The listing builds one solid part. Answer for the finished solid, in the listing's coordinates (mm). Face numbers are marked on the shaded views. Give positions to 0.01 mm unless a question says otherwise; leave off trailing zeros. Loops run counter-clockwise (first coordinate to the right, second up) from the corner with the lowest first, then second, coordinate; pieces in that order, holes last. Notation, with made-up numbers: M 69,17 L 76,17 A24 cw 76,56 Z; hole C 87,39.25 d2. An arc over 180 degrees is marked long. One line per item, written item: value. Start each with the question number.
Q1. A flat-ended cylindrical pin translates along its axis: pin 1 (4 mm diameter, centred on x = -9, y = 6.5, fed in from +Z). Find the tip coordinate at first contact, or state that the pin passes through.
Q2. A cutting plane is placed at D-D, the plane z = 3.15. Determine the outline of the cut face in (x, y) (3 decimals), and give its area (3 significant figures).
Q3. A cutting plane is placed at C-C, the plane y = 14. Determine the outline of the cut face in (x, z).
Q4. A cutting plane is placed at A-A, the plane y = 0. Determine the outline of the cut face in (x, z) (3 decimals).
Q5. Consider L1, parallel to Y at x = 0, z = 1.1 (3 decimals); L2, parallel to Y at x = 0, z = 3.2 (3 decimals); L3, parallel to X at y = 6, z = 1.55. Determine where each line is inside the solid, lowest interval first.
Q6. The mould has two halves that part along X. Classify the marked faces 1, 2 and 3: +X half, -X half, draft (parallel to the pull), parting line (faces both ways), or undercut.
Q7. A cutting plane is placed at B-B, the plane x = 0. Determine the outline of the cut face in (y, z) (3 decimals).
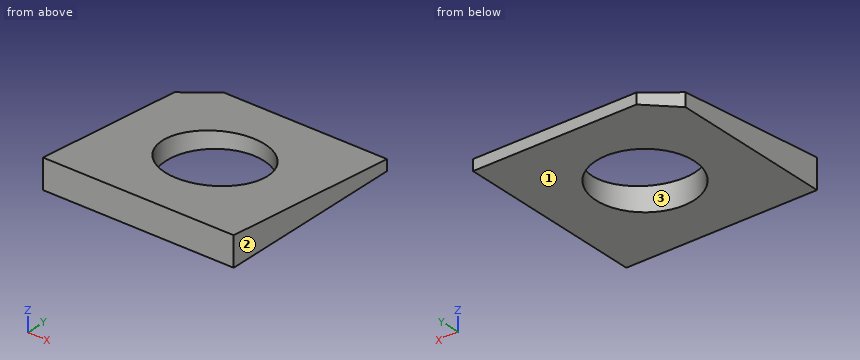
from build123d import *

# Parameters (mm, degrees)
SKETCH1_W          = 35
SKETCH1_H          = 35
SKETCH1_R          = 8.965
BOSS_EXTRUDE_DEPTH = 5.4
SKETCH2_OUTSIDE_W  = 17.358
SKETCH2_OUTSIDE_H  = 46.958
CUT_EXTRUDE1_DEPTH = 35
CUT_EXTRUDE2_DEPTH = 26.331008665


with BuildPart() as part:
    # Sketch1 → Boss-Extrude (new body)
    with BuildSketch(Plane.XY):
        Rectangle(SKETCH1_W, SKETCH1_H)
        with Locations(Location((0, 0, 0), (0, 0, 180))):
            Circle(SKETCH1_R, mode=Mode.SUBTRACT)
    extrude(amount=BOSS_EXTRUDE_DEPTH)

    # Sketch2 outside → Cut-Extrude1 (cut)
    with BuildSketch(Plane(origin=(17.5, 0, 0), x_dir=(0, 0, -1), z_dir=(1, 0, 0))):
        with Locations((-2.7, 0)):
            Rectangle(SKETCH2_OUTSIDE_W, SKETCH2_OUTSIDE_H)
        Polygon((-5.4, -17.5), (-2, 17.5), (0, 17.5), (0, -17.5), align=None, mode=Mode.SUBTRACT)
    extrude(amount=-CUT_EXTRUDE1_DEPTH, mode=Mode.SUBTRACT)

    # Sketch3 → Cut-Extrude2 (cut, through all)
    with BuildSketch(Plane(origin=(0, 0, 0), x_dir=(-1, 0, 0), z_dir=(0, 0, -1))):
        Polygon((12.5, 17.5), (17.5, 12.5), (17.5, 17.5), align=None)
    extrude(amount=-CUT_EXTRUDE2_DEPTH, mode=Mode.SUBTRACT)


solid = part.part
Answer block:
1. pin 1: z = 3.26
2. outline: M -17.5,-17.5 L 17.5,-17.5 L 17.5,5.662 L 6.951,5.662 A8.965 cw long -6.951,5.662 L -17.5,5.662 Z
2. area: 590 mm^2
3. outline: M -16,0 L 17.5,0 L 17.5,2.34 L -16,2.34 Z
4. outline: M -17.5,0 L -8.965,0 L -8.965,3.7 L -17.5,3.7 Z; M 8.965,0 L 17.5,0 L 17.5,3.7 L 8.965,3.7 Z
5. L1: -17.5 to -8.965, 8.965 to 17.5
5. L2: -17.5 to -8.965
5. L3: -17.5 to -6.66, 6.66 to 17.5
6. face 1: draft
6. face 2: +X half
6. face 3: undercut
7. outline: M -17.5,0 L -8.965,0 L -8.965,4.571 L -17.5,5.4 Z; M 8.965,0 L 17.5,0 L 17.5,2 L 8.965,2.829 Z
